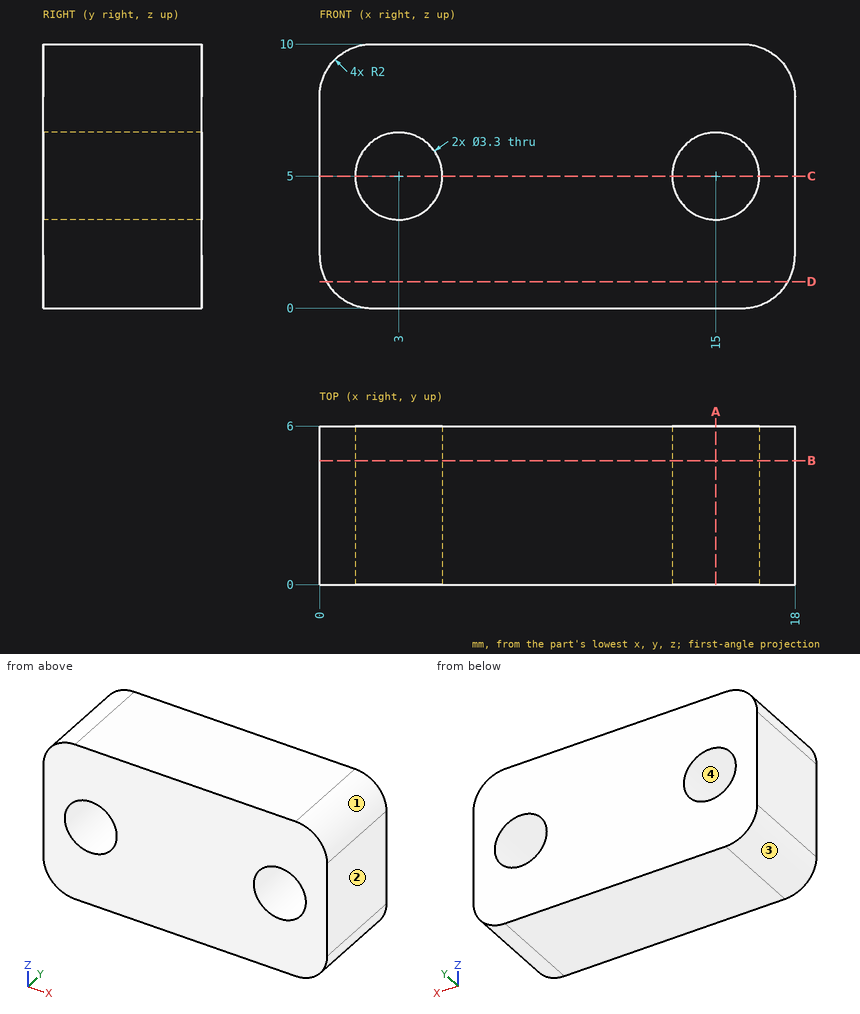
Job drawing, mm, ordinate dimensions from the low corner. One solid piece. Round coordinates to 2 decimals unless told otherwise and drop trailing zeros. Write each loop counter-clockwise with the first axis right and the second up, starting at its lowest first coordinate (ties: lowest second). Pieces come first, ordered by that corner, then holes.
1) Band-saw the part on D-D, the plane z = 1. List the corners of the cut face in (x, y), and give its area (3 significant figures).
2) Band-saw the part on A-A, the plane x = 15. List the corners of the cut face in (y, z).
3) Band-saw the part on B-B, the plane y = 4.7. List the corners of the cut face in (x, z), and give its area (3 significant figures).
4) Drill centre lines: probe 1 along X at (y, z) = (4, 5); probe 2 along Z at (x, y) = (3, 1.4); probe 3 along X at (y, z) = (3.25, 4). Where is each one in solid material? Low to high.
5) Mould opens along Z. For the marked faces 1, 2, 3 and 4 say: +Z half, -Z half, draft (parallel to the pull), parting line (faces both ways), or undercut.
6) Band-saw the part on C-C, the plane z = 5. List the corners of the cut face in (x, y).
Ans:
1. outline: (0.27, 0) - (17.73, 0) - (17.73, 6) - (0.27, 6) - close
1. area: 105 mm2
2. outline: (0, 0) - (6, 0) - (6, 3.35) - (0, 3.35) - close; (0, 6.65) - (6, 6.65) - (6, 10) - (0, 10) - close
3. outline: (0, 2) arc R2 ccw to (2, 0) - (16, 0) arc R2 ccw to (18, 2) - (18, 8) arc R2 ccw to (16, 10) - (2, 10) arc R2 ccw to (0, 8) - close; hole circle Ø3.3 at (3, 5); hole circle Ø3.3 at (15, 5)
3. area: 159 mm2
4. probe 1: x = 0 to 1.35, 4.65 to 13.35, 16.65 to 18
4. probe 2: z = 0 to 3.35, 6.65 to 10
4. probe 3: x = 0 to 1.69, 4.31 to 13.69, 16.31 to 18
5. face 1: +Z half
5. face 2: draft
5. face 3: -Z half
5. face 4: undercut
6. outline: (0, 0) - (1.35, 0) - (1.35, 6) - (0, 6) - close; (4.65, 0) - (13.35, 0) - (13.35, 6) - (4.65, 6) - close; (16.65, 0) - (18, 0) - (18, 6) - (16.65, 6) - close
